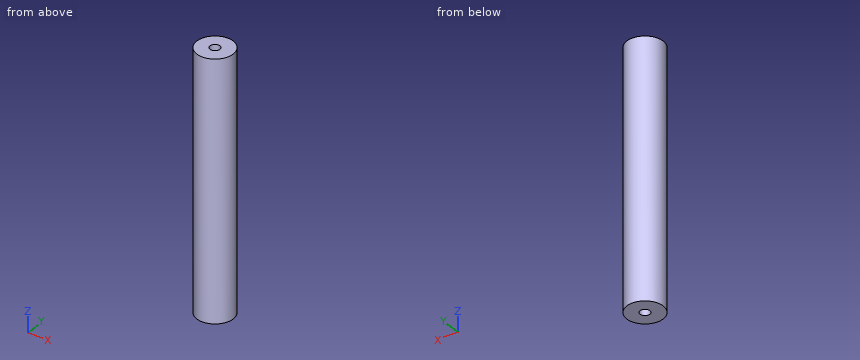
```python
from build123d import *

# Parameters (mm, degrees)
SKETCH_1_R             = 12.5
EXTRUDE_1_DEPTH        = 176
HOLE_WIZARD_M8_1_D     = 6.8
HOLE_WIZARD_M8_1_DEPTH = 19.75
HOLE_WIZARD_M8_1_TIP   = 2.042926105
HOLE_WIZARD_M8_2_D     = 6.8
HOLE_WIZARD_M8_2_DEPTH = 19.75
HOLE_WIZARD_M8_2_TIP   = 2.042926105


with BuildPart() as part:
    # 草图1 → 凸台-拉伸1 (new body)
    with BuildSketch(Plane.XY):
        Circle(SKETCH_1_R)
    extrude(amount=EXTRUDE_1_DEPTH)

    # M8 螺纹孔1
    with Locations(Plane(origin=(0, 0, 0), x_dir=(-1, 0, 0), z_dir=(0, 0, -1))):
        with Locations((0, 0)):
            Hole(HOLE_WIZARD_M8_1_D / 2, depth=HOLE_WIZARD_M8_1_DEPTH)
            with Locations((0, 0, -(HOLE_WIZARD_M8_1_DEPTH + HOLE_WIZARD_M8_1_TIP / 2))):  # 118° drill point
                Cone(0, HOLE_WIZARD_M8_1_D / 2, HOLE_WIZARD_M8_1_TIP, mode=Mode.SUBTRACT)

    # M8 螺纹孔2
    with Locations(Plane.XY.offset(176)):
        with Locations((0, 0)):
            Hole(HOLE_WIZARD_M8_2_D / 2, depth=HOLE_WIZARD_M8_2_DEPTH)
            with Locations((0, 0, -(HOLE_WIZARD_M8_2_DEPTH + HOLE_WIZARD_M8_2_TIP / 2))):  # 118° drill point
                Cone(0, HOLE_WIZARD_M8_2_D / 2, HOLE_WIZARD_M8_2_TIP, mode=Mode.SUBTRACT)


solid = part.part
```
Check sheet for the modelled part. Datum: model origin and axes. Units: mm. Give positions to 0.01 mm unless a question says otherwise; leave off trailing zeros. Order: outer loops, then holes, each group sorted by start corner. A loop starts at its lowest first (then second) coordinate and runs counter-clockwise, first axis right, second up. Notation, with made-up numbers: (81, 24) -> (112, 24) arc R20 ccw to (112, 39) -> close; hole circle Ø1 at (47.5, -16). An arc over 180 degrees is marked (long way). Return JSON: item names as keys, results as strings.
1. Cross-section at B-B, the plane x = -5. Record the cut outline in (y, z).
From the geometry:
{"outline": "(-11.46, 0) -> (11.46, 0) -> (11.46, 176) -> (-11.46, 176) -> close"}
2. Cross-section at A-A, the plane z = 99. Record the cut outline in (x, y).
From the geometry:
{"outline": "circle Ø25 at (0, 0)"}
3. Cross-section at C-C, the plane y = -8.75. Record the cut outline in (x, z), plus the area to 3 significant figures.
From the geometry:
{"outline": "(-8.93, 0) -> (8.93, 0) -> (8.93, 176) -> (-8.93, 176) -> close", "area": "3,140 mm^2"}
4. Material ranges on probe 1 along Y at (x, z) = (0, 14.75); probe 2 along Y at (x, z) = (0.75, 93.5); probe 3 along X at (y, z) = (-0.5, 39), recorded low to high. Write a range as [from, to].
From the geometry:
{"probe 1": "[-12.5, -3.4], [3.4, 12.5]", "probe 2": "[-12.48, 12.48]", "probe 3": "[-12.49, 12.49]"}
5. Go/stop test with flat-tipped pins: P1, Ø1.5, axis at y = -6, z = 151, coming from the +X side; P2, Ø2, axis at y = -6.5, z = 89.5, coming from the +X side (3 decimals); P3, Ø12, axis at x = 8.5, z = 66, coming from the +Y side. Record where each tip stops, or that it passes through.
From the geometry:
{"P1": "x = 11.34", "P2": "x = 11.225", "P3": "y = 12.25"}
